Verification items for the finished model (mm, model axes). A direction names the side the tool comes from. Coordinates: 2 decimals unless noted, no trailing zeros. Order: outer loops, then holes, each group sorted by start corner. A loop starts at its lowest first (then second) coordinate and runs counter-clockwise, first axis right, second up. Notation, with made-up numbers: M -2.5,-36 L 24.5,-36 A18 ccw 24.5,-10 Z; hole C 18.5,24 d11. An arc over 180 degrees is marked long. Write item = value, one per line.
```python
from build123d import *

# Parameters (mm, degrees)
BOSS_EXTRUDE1_DEPTH = 10


with BuildPart() as part:
    # Sketch1 → Boss-Extrude1 (new body)
    with BuildSketch(Plane(origin=(0, 0, 0), x_dir=(1, 0, 0), z_dir=(0, 1, 0))):
        Polygon((0, 0), (4, 0), (4, -7), (14, -7), (14, -4), (7, -4), (7, 3), (0, 3), align=None)
    extrude(amount=BOSS_EXTRUDE1_DEPTH)


solid = part.part
```
Item 1: Sectioned sample at B-B, the plane z = -0.5. Enter the section's corners in (x, y).
Report:
outline = M 0,0 L 7,0 L 7,10 L 0,10 Z
Item 2: Scan lines: L1, parallel to Z at x = 7.25, y = 4.25; L2, parallel to Z at x = 1, y = 8. Record each from-to range of solid material in increasing order. Write a range as from..to.
Report:
L1 = 4..7
L2 = -3..0
Item 3: Tool access check on faces 1 (the flat face through (11, 5, 4)), 2 (the flat face through (2, 5, 0)), 3 (the flat face through (14, 5, 6)). Record the directions out of +Z, -Z, +X, -X, +Y, -Y that give a thin tool (end or side, any length) a straight path to the whole face; none if there is none.
Report:
face_1 = -Z, +X, +Y, -Y
face_2 = +Z, -X, +Y, -Y
face_3 = +Z, -Z, +X, +Y, -Y
Item 4: Sectioned sample at A-A, the plane y = 2.5. Enter the section's corners in (x, z).
Report:
outline = M 0,-3 L 7,-3 L 7,4 L 14,4 L 14,7 L 4,7 L 4,0 L 0,0 Z
Item 5: Sectioned sample at C-C, the plane x = 7.5. Enter the section's corners in (y, z), then the cut area to 3 significant figures.
Report:
outline = M 0,4 L 10,4 L 10,7 L 0,7 Z
area = 30.0 mm^2
Item 6: Gauge pin test, flat ends, axial feed: pin 1 (2 mm diameter, centred on y = 7, z = 0.5, fed in from +X); pin 2 (6 mm diameter, centred on y = 5, z = 5, fed in from -X); pin 3 (3 mm diameter, centred on x = 2, y = 7.5, fed in from +Z). Record the tip position at first contact, or that the pin passes through.
Report:
pin_1 = 7
pin_2 = 4
pin_3 = 0
